Verification items for the finished model (mm, model axes). A direction names the side the tool comes from. Give positions to 0.01 mm unless a question says otherwise; leave off trailing zeros. Write each loop counter-clockwise with the first axis right and the second up, starting at its lowest first coordinate (ties: lowest second). Pieces come first, ordered by that corner, then holes. Notation, with made-up numbers: (-3.75, 48.25) - (20.25, 48.25) arc R15 cw to (20.25, 77.25) - close; hole circle Ø2 at (-29.5, 39). An arc over 180 degrees is marked (long way). Put each result on its own line as item: value.
from build123d import *

# Parameters (mm, degrees)
SKETCH_2_R                = 13.5
CUT_EXTRUDE_M28_1_0_DEPTH = 300


with BuildPart() as part:
    # 草图1 → 旋转1 (revolve)
    with BuildSketch(Plane.XY, mode=Mode.PRIVATE) as revolve_1_sk:
        Polygon((0, 0), (0, 15), (120, 15), (120, 22), (150, 22), (150, 19), (190, 19), (190, 22), (220, 22), (220, 15), (400, 15), (400, 0), align=None)
    revolve(revolve_1_sk.sketch.rotate(Axis((0, 0, 0), (1, 0, 0)), 90), axis=Axis((0, 0, 0), (1, 0, 0)))

    # 草图2 → 螺纹孔M28*1.0 (cut)
    with BuildSketch(Plane.ZY):
        Circle(SKETCH_2_R)
    extrude(amount=-CUT_EXTRUDE_M28_1_0_DEPTH, mode=Mode.SUBTRACT)


solid = part.part
Q1. Section check B-B, the plane z = 6.5. Record the cut outline in (x, y).
Answers follow:
outline: (0, -13.52) - (120, -13.52) - (120, -21.02) - (150, -21.02) - (150, -17.85) - (190, -17.85) - (190, -21.02) - (220, -21.02) - (220, -13.52) - (400, -13.52) - (400, 13.52) - (220, 13.52) - (220, 21.02) - (190, 21.02) - (190, 17.85) - (150, 17.85) - (150, 21.02) - (120, 21.02) - (120, 13.52) - (0, 13.52) - (0, 11.83) - (300, 11.83) - (300, -11.83) - (0, -11.83) - close
Q2. Section check C-C, the plane y = 0. Record the cut outline in (x, z), plus the area to 3 significant figures.
Answers follow:
outline: (0, -15) - (120, -15) - (120, -22) - (150, -22) - (150, -19) - (190, -19) - (190, -22) - (220, -22) - (220, -15) - (400, -15) - (400, 15) - (220, 15) - (220, 22) - (190, 22) - (190, 19) - (150, 19) - (150, 22) - (120, 22) - (120, 15) - (0, 15) - (0, 13.5) - (300, 13.5) - (300, -13.5) - (0, -13.5) - close
area: 5,060 mm2
Q3. Set-up check for faces 1 (the face through (0, -7.85, 11.18)), 2 (the face through (311.26, -12.65, 8.06)), 3 (the face through (190, -18, 7)), 4 (the face through (205.21, 21.477, -4.769)), 5 (the face through (120, -5.2, -14.4)): record each of +Z, -Z, +X, -X, +Y, -Y from which the full face is reachable in a straight line by a thin tool's end or side.
Answers follow:
face 1: +Z, -Z, -X, +Y, -Y
face 2: +X
face 3: none
face 4: +X, -X
face 5: -X
Q4. Go/stop test with flat-tipped pins: pin 1 Ø4 at (x, z) = (304.5, -9) entering from +Y; pin 2 Ø1 at (x, y) = (293, 10.5) entering from -Z; pin 3 Ø2 at (x, y) = (275, 11) entering from +Z. Record where each tip stops, or that it passes through.
Answers follow:
pin 1: stops at y = 13.27
pin 2: stops at z = -11.18
pin 3: stops at z = 11.18
Q5. Section check A-A, the plane x = 294. Record the cut outline in (y, z), plus the area to 3 significant figures.
Answers follow:
outline: circle Ø30 at (0, 0); hole circle Ø27 at (0, 0)
area: 134 mm2
Q6. Release check for a two-part mould opening along Y. For faces 6 (the face through (170.28, 18.548, -4.119)), 7 (the face through (300, 0, 0)), 8 (the face through (150, -18, -7)) record: released by +Y, released by -Y, zero draft, split by the parting line, or undercut.
Answers follow:
face 6: split by the parting line
face 7: undercut
face 8: zero draft
Q7. Section check D-D, the plane x = 128.5. Record the cut outline in (y, z).
Answers follow:
outline: circle Ø44 at (0, 0); hole circle Ø27 at (0, 0)
Q8. Scan lines: line 1 along Y through (x, z) = (162, 0); line 2 along X through (y, z) = (16, -13); line 3 along Y through (x, z) = (200.5, 1). Record each from-to range of solid material in increasing order.
Answers follow:
line 1: y = -19 to -13.5, 13.5 to 19
line 2: x = 120 to 150, 190 to 220
line 3: y = -21.98 to -13.46, 13.46 to 21.98
